```python
from build123d import *

# Parameters (mm, degrees)
BOSS_EXTRUDE1_DEPTH = 6.4
SKETCH3_R           = 5
BOSS_EXTRUDE2_DEPTH = 35
CHAMFER1_SIZE       = 1


with BuildPart() as part:
    # Sketch1 → Boss-Extrude1 (new body)
    with BuildSketch(Plane.XY):
        Polygon((8, 4.618802154), (0, 9.237604307), (-8, 4.618802154), (-8, -4.618802154), (0, -9.237604307), (8, -4.618802154), align=None)
    extrude(amount=BOSS_EXTRUDE1_DEPTH)

    # Sketch3 → Boss-Extrude2 (add)
    with BuildSketch(Plane.XY.offset(6.4)):
        Circle(SKETCH3_R)
    extrude(amount=BOSS_EXTRUDE2_DEPTH)

    # Chamfer1
    chamfer1_edges = [part.edges().sort_by_distance(p)[0] for p in [
        (-5, 0, 41.4),
    ]]
    chamfer(chamfer1_edges, length=CHAMFER1_SIZE)


solid = part.part
```
Part model, mm, in its own coordinate system. A direction names the side the tool comes from. Coordinates: 2 decimals unless noted, no trailing zeros. Order: outer loops, then holes, each group sorted by start corner. A loop starts at its lowest first (then second) coordinate and runs counter-clockwise, first axis right, second up. Notation, with made-up numbers: (41.25, -22) - (85.25, -22) arc R7 ccw to (85.25, -17) - close; hole circle Ø9 at (-22, -23). An arc over 180 degrees is marked (long way). Return JSON: item names as keys, results as strings. Group by question number.
Item 1: Pin check, flat tips, straight feed: pin 1 (8 mm diameter, centred on x = 3.5, z = 23.5, fed in from +Y); pin 2 (8 mm diameter, centred on y = -6, z = 24, fed in from +X); pin 3 (6 mm diameter, centred on y = 3.5, z = 14, fed in from +X); pin 4 (10 mm diameter, centred on y = -7, z = 10.5, fed in from +X). Stop position of each tip, or through.
Item 2: Cut at D-D (y = 7.25). List the corners of the cut face in (x, z).
Item 3: Cut at A-A (y = 0). List the corners of the cut face in (x, z), plus the area to 3 significant figures.
Item 4: Drill centre lines: probe 1 along Z at (x, y) = (-1, 6.5); probe 2 along X at (y, z) = (-7, 6); probe 3 along Z at (x, y) = (2.5, -3.75). Where is each one in solid material? Low to high. Write a range as from..to.
Item 5: Cut at C-C (z = 23). List the corners of the cut face in (x, y).
Item 6: Cut at B-B (z = 4). List the corners of the cut face in (x, y), plus the area to 3 significant figures.
Item 7: Which spindle directions (+Z, -Z, +X, -X, +Y, -Y) get a long thin tool onto all of the face, cutting with end or side? Do faces 1 (the face through (-8, 0, 3)), 2 (the face through (3.4, -4, 6.4)). Say none if no direction does.
Check values:
{
 "1": {"pin 1": "stops at y = 5", "pin 2": "stops at x = 4.58", "pin 3": "stops at x = 4.97", "pin 4": "stops at x = 8"},
 "2": {"outline": "(-3.44, 0) - (3.44, 0) - (3.44, 6.4) - (-3.44, 6.4) - close"},
 "3": {"outline": "(-8, 0) - (8, 0) - (8, 6.4) - (5, 6.4) - (5, 40.4) - (4, 41.4) - (-4, 41.4) - (-5, 40.4) - (-5, 6.4) - (-8, 6.4) - close", "area": "451 mm2"},
 "4": {"probe 1": "z = 0..6.4", "probe 2": "x = -3.88..3.88", "probe 3": "z = 0..40.89"},
 "5": {"outline": "circle Ø10 at (0, 0)"},
 "6": {"outline": "(-8, -4.62) - (0, -9.24) - (8, -4.62) - (8, 4.62) - (0, 9.24) - (-8, 4.62) - close", "area": "222 mm2"},
 "7": {"face 1": "+Z, -Z, -X, +Y, -Y", "face 2": "+Z"}
}
